Here's how the part is built. I have some questions about the finished solid (model axes, mm). A direction names the side the tool comes from. Round coordinates to 2 decimals unless told otherwise and drop trailing zeros. Write each loop counter-clockwise with the first axis right and the second up, starting at its lowest first coordinate (ties: lowest second). Pieces come first, ordered by that corner, then holes. Notation, with made-up numbers: (9, 69) -> (61, 69) arc R14 ccw to (61, 89) -> close; hole circle Ø7 at (-0.75, -22). An arc over 180 degrees is marked (long way). Answer as CSV lines item,"result".
from build123d import *

# Parameters (mm, degrees)
BASE_SADDLE_DEPTH          = 25
BASE_CORNER_FILLET_R14_R   = 14
PIN_BOSS_SKETCH_R          = 8
PIVOT_PIN_BOSS_16_DEPTH    = 14
PIN_BOSS_BORE_SKETCH_R     = 6
PIN_BOSS_BORE_12_DEPTH     = 86.638776264
PIN_BOSS_ROOT_FILLET_R3_R  = 3
CLEVIS_UPRIGHT_DEPTH       = 14
EYE_BOSS_SKETCH_R          = 19
EYE_BOSS_DEPTH             = 14
EYE_BORE_SKETCH_R          = 14
EYE_BORE_28_DEPTH          = 127.039676293
SADDLE_START               = -11
SADDLE_CLEARANCE_CUT_DEPTH = 11
SADDLE_RELIEF_CUT_DEPTH    = 11
CLEVIS_SLOT_SKETCH_W       = 12
CLEVIS_SLOT_SKETCH_H       = 38
CLEVIS_SLOT_12_DEPTH       = 12


with BuildPart() as part:
    # Base Saddle Profile Sketch → Base Saddle (new, symmetric)
    with BuildSketch(Plane(origin=(0, 0, 0), x_dir=(0, 0, -1), z_dir=(1, 0, 0))):
        with BuildLine():
            Line((23, 0), (78, 0))
            Line((78, 0), (78, 11))
            Line((78, 11), (34.278273002, 11))
            ThreePointArc((34.278273002, 11), (-5.566963801, 35.566963801), (-36, 0))
            Line((-36, 0), (-23, 0))
            ThreePointArc((-23, 0), (0, 23), (23, 0))
        make_face()
    extrude(amount=BASE_SADDLE_DEPTH, both=True)

    # Base Corner Fillet R14
    base_corner_fillet_r14_edges = [part.edges().sort_by_distance(p)[0] for p in [
        (25, 5.5, -78),
        (-25, 5.5, -78),
    ]]
    fillet(base_corner_fillet_r14_edges, radius=BASE_CORNER_FILLET_R14_R)

    # Pin Boss Sketch → Pivot Pin Boss Ø16 (add)
    with BuildSketch(Plane(origin=(0, 11, 0), x_dir=(1, 0, 0), z_dir=(0, 1, 0))):
        with Locations(Location((0, 59, 0), (0, 0, 90))):
            Circle(PIN_BOSS_SKETCH_R)
    extrude(amount=PIVOT_PIN_BOSS_16_DEPTH)

    # Pin Boss Bore Sketch → Pin Boss Bore Ø12 (cut, through all)
    with BuildSketch(Plane(origin=(0, 25, 0), x_dir=(1, 0, 0), z_dir=(0, 1, 0))):
        with Locations(Location((0, 59, 0), (0, 0, 270))):
            Circle(PIN_BOSS_BORE_SKETCH_R)
    extrude(amount=-PIN_BOSS_BORE_12_DEPTH, mode=Mode.SUBTRACT)

    # Pin Boss Root Fillet R3
    pin_boss_root_fillet_r3_edges = [part.edges().sort_by_distance(p)[0] for p in [
        (0, 11, -34.278273002),
        (0, 11, -51),
    ]]
    fillet(pin_boss_root_fillet_r3_edges, radius=PIN_BOSS_ROOT_FILLET_R3_R)

    # Clevis Upright Sketch → Clevis Upright (add, symmetric)
    with BuildSketch(Plane(origin=(0, 0, 0), x_dir=(0, 0, -1), z_dir=(1, 0, 0))):
        with BuildLine():
            Line((-36, 0), (-36, 72))
            Line((-36, 72), (2, 72))
            Line((2, 72), (2, 35.944401511))
            ThreePointArc((2, 35.944401511), (-24.738633754, 26.153393661), (-36, 0))
        make_face()
    extrude(amount=CLEVIS_UPRIGHT_DEPTH, both=True)

    # Eye Boss Sketch → Eye Boss (add, symmetric)
    with BuildSketch(Plane(origin=(0, 0, 0), x_dir=(0, 0, -1), z_dir=(1, 0, 0))):
        with Locations((-17, 72)):
            Circle(EYE_BOSS_SKETCH_R)
    extrude(amount=EYE_BOSS_DEPTH, both=True)

    # Eye Bore Sketch → Eye Bore Ø28 (cut, through all)
    with BuildSketch(Plane.ZY.offset(14)):
        with Locations((17, 72)):
            Circle(EYE_BORE_SKETCH_R)
    extrude(amount=-EYE_BORE_28_DEPTH, mode=Mode.SUBTRACT)

    # Saddle Clearance Sketch → Saddle Clearance Cut (cut)
    with BuildSketch(Plane.ZY.offset(25).offset(SADDLE_START)):
        with BuildLine():
            Line((-19.899748742, 30), (19.899748742, 30))
            ThreePointArc((19.899748742, 30), (0, 36), (-19.899748742, 30))
        make_face()
    extrude(amount=SADDLE_CLEARANCE_CUT_DEPTH, mode=Mode.SUBTRACT)

    # Saddle Relief Sketch → Saddle Relief Cut (cut)
    with BuildSketch(Plane(origin=(25, 0, 0), x_dir=(0, 0, -1), z_dir=(1, 0, 0))):
        with BuildLine():
            Line((19.899748742, 30), (-19.899748742, 30))
            ThreePointArc((-19.899748742, 30), (0, 36), (19.899748742, 30))
        make_face()
    extrude(amount=-SADDLE_RELIEF_CUT_DEPTH, mode=Mode.SUBTRACT)

    # Clevis Slot Sketch → Clevis Slot 12 (cut)
    with BuildSketch(Plane(origin=(0, 91, 0), x_dir=(-1, 0, 0), z_dir=(0, -1, 0))):
        with Locations((0, -17)):
            Rectangle(CLEVIS_SLOT_SKETCH_W, CLEVIS_SLOT_SKETCH_H)
    extrude(amount=CLEVIS_SLOT_12_DEPTH, mode=Mode.SUBTRACT)


solid = part.part
Item 1: Will these pins go through, and if not, where does the flat tip stop? pin 1 (1 mm diameter, centred on y = 30, z = 24, fed in from -X); pin 2 (4 mm diameter, centred on x = 14, y = 34, fed in from -Z); pin 3 (17.5 mm diameter, centred on x = 3.5, z = -61.5, fed in from +Y).
Results found:
pin 1,"stops at x = -14"
pin 2,"stops at z = -16.49"
pin 3,"stops at y = 25"
Item 2: I need wall thicknesses on L1, parallel to X at y = 19, z = -59; L2, parallel to Y at x = -15, z = -57; L3, parallel to Y at x = -7.5, z = 6.5. Which ranges of each line are inside material? Lowest first, please.
Results found:
L1,"x = -8 to -6, 6 to 8"
L2,"y = 0 to 11"
L3,"y = 22.06 to 62.74, 81.26 to 87.84"
Item 3: For faces 1 (the flat face through (0, 54, -2)), 2 (the flat face through (0, 79, 2)), 3 (the cylindrical face through (19.577, 17.242, 31.602)), 4 (the flat face through (-19, 30, 0)), which set-ups out of +Z, -Z, +X, -X, +Y, -Y let a thin tool reach every point of the face, with its end or its side?
Results found:
face 1,"-Z, +X, -X, +Y"
face 2,"+Z, -Z, +Y"
face 3,"+Z, +X, +Y"
face 4,"+Z, -Z, -X, +Y"
Item 4: Suppose I cut it at D-D, the plane z = 7. List the corners of the cut face in (x, y) for me, then the cut area to 3 significant figures.
Results found:
outline,"(-25, 21.91) -> (25, 21.91) -> (25, 30) -> (14, 30) -> (14, 62.2) -> (-14, 62.2) -> (-14, 30) -> (-25, 30) -> close; (-14, 81.8) -> (-6, 81.8) -> (-6, 88.16) -> (-14, 88.16) -> close; (6, 81.8) -> (14, 81.8) -> (14, 88.16) -> (6, 88.16) -> close"
area,"1,410 mm²"
Item 5: Suppose I cut it at A-A, the plane x = 0. List the corners of the cut face in (y, z) for me.
Results found:
outline,"(0, -78) -> (11, -78) -> (11, -70) arc R3 cw to (14, -67) -> (25, -67) -> (25, -65) -> (0, -65) -> close; (0, -53) -> (25, -53) -> (25, -51) -> (14, -51) arc R3 cw to (11, -48) -> (11, -36.4) arc R3 cw to (12.92, -33.6) arc R36 ccw to (35.94, -2) -> (72, -2) arc R19 ccw to (79, -0.66) -> (79, 4.88) arc R14 cw (long way) to (79, 29.12) -> (79, 34.66) arc R19 ccw to (72, 36) -> (0, 36) -> (0, 23) arc R23 cw to (0, -23) -> close"
Item 6: Suppose I cut it at C-C, the plane y = 20.5. List the corners of the cut face in (x, z) for me.
Results found:
outline,"(-25, -29.59) -> (25, -29.59) -> (25, -10.43) -> (-25, -10.43) -> close; (-25, 10.43) -> (25, 10.43) -> (25, 29.59) -> (14, 29.59) -> (14, 36) -> (-14, 36) -> (-14, 29.59) -> (-25, 29.59) -> close; circle Ø16 at (0, -59); hole circle Ø12 at (0, -59)"
Item 7: If we mould it in two halves opening along X, with no side actions, what happens to faces 5 (the flat face through (6, 86.4, 17.2)), 6 (the flat face through (14, 49, 19)), 7 (the flat face through (0, 0, 30))? For each: pulls with the +X half, pulls with the -X half, needs draft (parallel to the pull), parting line crosses it, or undercut.
Results found:
face 5,"undercut"
face 6,"pulls with the +X half"
face 7,"needs draft"
Item 8: Suppose I cut it at B-B, the plane z = -59. List the corners of the cut face in (x, y) for me, then the cut area to 3 significant figures.
Results found:
outline,"(-25, 0) -> (-6, 0) -> (-6, 25) -> (-8, 25) -> (-8, 14) arc R3 cw to (-11, 11) -> (-25, 11) -> close; (6, 0) -> (25, 0) -> (25, 11) -> (11, 11) arc R3 cw to (8, 14) -> (8, 25) -> (6, 25) -> close"
area,"478 mm²"
